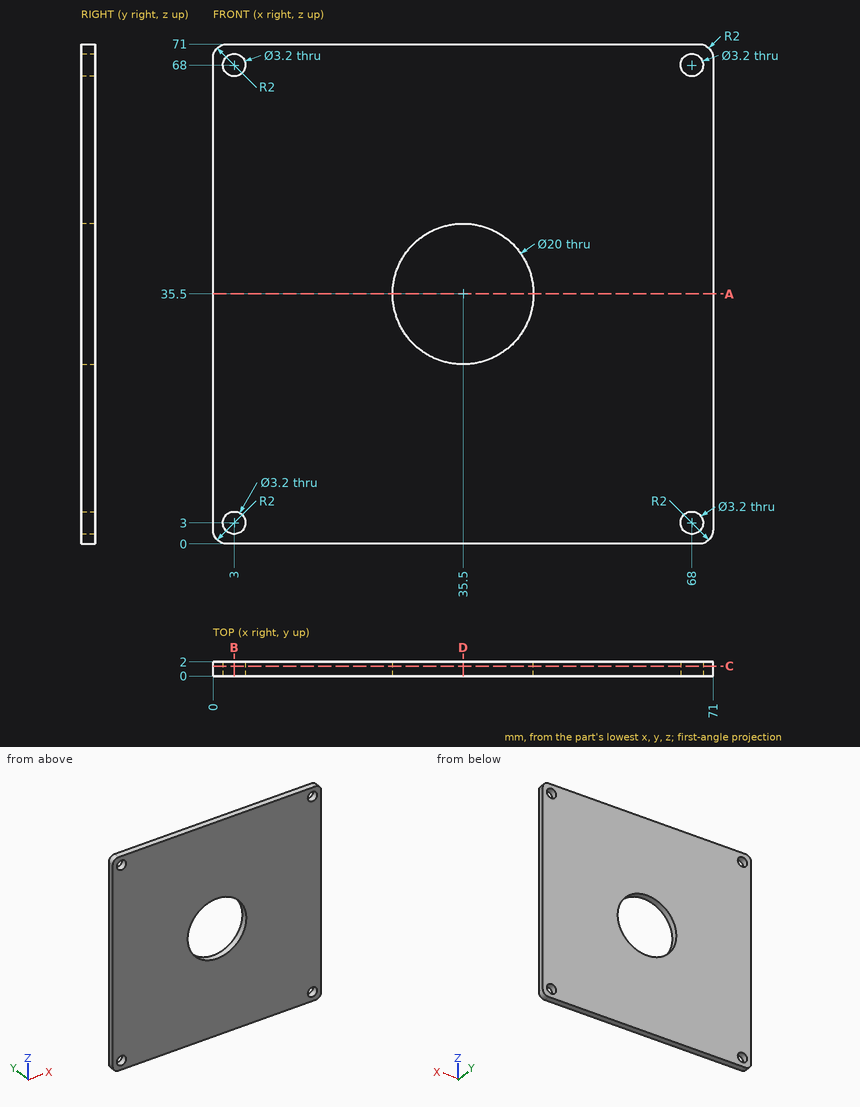
Part print with two shaded views. Sizes in mm from the minimum x, y, z corner. Give positions to 0.01 mm unless a question says otherwise; leave off trailing zeros. Order: outer loops, then holes, each group sorted by start corner. A loop starts at its lowest first (then second) coordinate and runs counter-clockwise, first axis right, second up.
(1) Saw through at B-B, the plane x = 3. Give the cut face in (y, z), then the cut area to 3 significant figures.
(2) Saw through at A-A, the plane z = 35.5. Give the cut face in (x, y).
(3) Saw through at D-D, the plane x = 35.5. Give the cut face in (y, z), then the cut area to 3 significant figures.
(4) Drill centre lines: L1, parallel to X at y = 0.85, z = 68; L2, parallel to Z at x = 67.5, y = 0.85. Where is each one in solid material? Low to high.
(5) Saw through at C-C, the plane y = 1.4. Give the cut face in (x, z).
Results found:
1. outline: (0, 0) - (2, 0) - (2, 1.4) - (0, 1.4) - close; (0, 4.6) - (2, 4.6) - (2, 66.4) - (0, 66.4) - close; (0, 69.6) - (2, 69.6) - (2, 71) - (0, 71) - close
1. area: 129 mm2
2. outline: (0, 0) - (25.5, 0) - (25.5, 2) - (0, 2) - close; (45.5, 0) - (71, 0) - (71, 2) - (45.5, 2) - close
3. outline: (0, 0) - (2, 0) - (2, 25.5) - (0, 25.5) - close; (0, 45.5) - (2, 45.5) - (2, 71) - (0, 71) - close
3. area: 102 mm2
4. L1: x = 0 to 1.4, 4.6 to 66.4, 69.6 to 71
4. L2: z = 0 to 1.48, 4.52 to 66.48, 69.52 to 71
5. outline: (0, 2) arc R2 ccw to (2, 0) - (69, 0) arc R2 ccw to (71, 2) - (71, 69) arc R2 ccw to (69, 71) - (2, 71) arc R2 ccw to (0, 69) - close; hole circle Ø3.2 at (3, 3); hole circle Ø3.2 at (3, 68); hole circle Ø20 at (35.5, 35.5); hole circle Ø3.2 at (68, 3); hole circle Ø3.2 at (68, 68)
